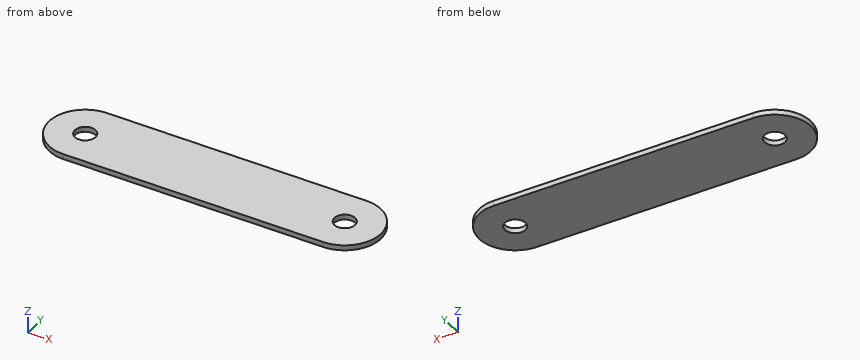
```python
from build123d import *

# Parameters (mm, degrees)
SKETCH1_R           = 2
BOSS_EXTRUDE1_DEPTH = 1


with BuildPart() as part:
    # Sketch1 → Boss-Extrude1 (new body)
    with BuildSketch(Plane.XY):
        with BuildLine():
            Line((-33.139059677, 7), (16.860940323, 7))
            ThreePointArc((16.860940323, 7), (23.860940323, 0), (16.860940323, -7))
            Line((16.860940323, -7), (-33.139059677, -7))
            ThreePointArc((-33.139059677, -7), (-40.139059677, 0), (-33.139059677, 7))
        make_face()
        with Locations((-33.139059677, 0)):
            Circle(SKETCH1_R, mode=Mode.SUBTRACT)
        with Locations((16.860940323, 0)):
            Circle(SKETCH1_R, mode=Mode.SUBTRACT)
    extrude(amount=BOSS_EXTRUDE1_DEPTH)


solid = part.part
```
The model under review builds one solid part; all positions refer to its coordinate system, in mm. Coordinates: 2 decimals unless noted, no trailing zeros. Order: outer loops, then holes, each group sorted by start corner. A loop starts at its lowest first (then second) coordinate and runs counter-clockwise, first axis right, second up. Notation, with made-up numbers: (61.5, 56) -> (81.5, 56) arc R26 ccw to (81.5, 76) -> close; hole circle Ø5 at (63.25, 10.25). An arc over 180 degrees is marked (long way). Answer in a Markdown table with one row per item. Add a question column.
Item 1: We need section A-A on y = 0. Write out the cut boundary in (x, z).
Item 2: To check wall thickness, follow probe 1 along X at (y, z) = (1.25, 0.75); probe 2 along X at (y, z) = (-0.75, 0.2); probe 3 along X at (y, z) = (-2.75, 0.9). State the ranges of each line that lie inside material, in increasing order.
Item 3: We need section B-B on z = 0.3. Write out the cut boundary in (x, y).
Item 4: Clearance check with flat-ended pins moving along their axes: pin 1 (5 mm diameter, centred on x = -11.5, y = 5.5, fed in from -Z); pin 2 (3.5 mm diameter, centred on x = -33.14, y = 0, fed in from +Z). State where each tip first meets the part, or that it passes through.
Item 5: We need section C-C on y = 2.75. Write out the cut boundary in (x, z), plus the area to 3 significant figures.
Final values:
| question | item | result |
|---|---|---|
| 1 | outline | (-40.14, 0) -> (-35.14, 0) -> (-35.14, 1) -> (-40.14, 1) -> close; (-31.14, 0) -> (14.86, 0) -> (14.86, 1) -> (-31.14, 1) -> close; (18.86, 0) -> (23.86, 0) -> (23.86, 1) -> (18.86, 1) -> close |
| 2 | probe 1 | x = -40.03 to -34.7, -31.58 to 15.3, 18.42 to 23.75 |
| 2 | probe 2 | x = -40.1 to -34.99, -31.29 to 15.01, 18.71 to 23.82 |
| 2 | probe 3 | x = -39.58 to 23.3 |
| 3 | outline | (-33.14, -7) -> (16.86, -7) arc R7 ccw to (16.86, 7) -> (-33.14, 7) arc R7 ccw to start; hole circle Ø4 at (-33.14, 0); hole circle Ø4 at (16.86, 0) |
| 4 | pin 1 | stops at z = 0 |
| 4 | pin 2 | passes through |
| 5 | outline | (-39.58, 0) -> (23.3, 0) -> (23.3, 1) -> (-39.58, 1) -> close |
| 5 | area | 62.9 mm2 |
